Design review of the part built by this model. Coordinates are the model's own, in mm. A direction names the side the tool comes from. Give positions to 0.01 mm unless a question says otherwise; leave off trailing zeros. Loops run counter-clockwise (first coordinate to the right, second up) from the corner with the lowest first, then second, coordinate; pieces in that order, holes last. Notation, with made-up numbers: (50.5, -8) -> (101.5, -8) arc R17 cw to (101.5, 14) -> close; hole circle Ø7 at (-17.5, 6). An arc over 180 degrees is marked (long way). Use a Markdown table: item, result. Add a question column.
1. Add section B-B (x = -83). State the section outline as (y, z) points, and give its area (3 significant figures).
2. To check wall thickness, follow line 1 (X direction, y = 2.5, z = -6); line 2 (Y direction, x = -66, z = -6.5); line 3 (Y direction, x = -9, z = -10). State the ranges of each line that lie inside material, in increasing order.
3. Add section C-C (y = 19). State the section outline as (x, z) points, and give its area (3 significant figures).
4. Add section A-A (z = 3.5). State the section outline as (x, y) points, and give its area (3 significant figures).
5. Draft analysis for pull direction X (two halves, no side actions). For faces 4 (the cylindrical face through (-99.1, 5.07, -20.14)), 5 (the cylindrical face through (-82.85, 11.97, -16.5)), 6 (the flat face through (-22.36, 32.38, 14.82)), state which applies: pulls with the +X half, pulls with the -X half, needs draft (parallel to the pull), parting line crosses it, or undercut.
6. For pin 1 Ø3 at (y, z) = (12, 2.5) entering from -X; pin 2 Ø11 at (x, z) = (-82, -3) entering from +Y; pin 3 Ø1.2 at (y, z) = (11.5, -1.5) entering from +X, all flat-tipped, find the tip position at first contact; note any pin that passes through.
7. Add section D-D (x = -19.5). State the section outline as (y, z) points, and give its area (3 significant figures).
8. For faces 1 (the cylindrical face through (-83.15, 11.97, 16.5)), 2 (the flat face through (-22.36, 29.612, 9.962)), 3 (the flat face through (-90, 12, 0)), list the 3-axis set-ups (+Z, -Z, +X, -X, +Y, -Y) from which the entire face can be reached by the end or side of a thin tool; tool diameter is ignored.
```python
from build123d import *

# Parameters (mm, degrees)
BASE_BLOCK_DEPTH         = 21
SLOT_BOSS_DEPTH          = 4
MOUNTING_START           = -34
MOUNTING_SLOT_DEPTH      = 34
DOVETAIL_GROOVE_55_DEPTH = 464
EDGE_FILLET_R3_R         = 3


with BuildPart() as part:
    # Base Profile Sketch → Base Block (new, symmetric)
    with BuildSketch(Plane.XY):
        Polygon((0, 0), (-100, 0), (-100, 10), (-60, 10), (-60, 31), (-44.102715558, 50.294464164), (0, 22.736028876), align=None)
    extrude(amount=BASE_BLOCK_DEPTH, both=True)

    # Slot Boss Sketch → Slot Boss (add)
    with BuildSketch(Plane(origin=(0, 10, 0), x_dir=(1, 0, 0), z_dir=(0, 1, 0))):
        with BuildLine():
            Line((-90, 9.5), (-90, -9.5))
            ThreePointArc((-90, -9.5), (-83, -16.5), (-76, -9.5))
            Line((-76, -9.5), (-76, 9.5))
            ThreePointArc((-76, 9.5), (-83, 16.5), (-90, 9.5))
        make_face()
        with BuildLine():
            Line((-88, 9.5), (-88, -9.5))
            ThreePointArc((-88, -9.5), (-83, -14.5), (-78, -9.5))
            Line((-78, -9.5), (-78, 9.5))
            ThreePointArc((-78, 9.5), (-83, 14.5), (-88, 9.5))
        make_face(mode=Mode.SUBTRACT)
    extrude(amount=SLOT_BOSS_DEPTH)

    # Mounting Slot Sketch → Mounting Slot (cut)
    with BuildSketch(Plane(origin=(0, 10, 0), x_dir=(1, 0, 0), z_dir=(0, 1, 0)).offset(MOUNTING_START)):
        with BuildLine():
            Line((-88, 9.5), (-88, -9.5))
            ThreePointArc((-88, -9.5), (-83, -14.5), (-78, -9.5))
            Line((-78, -9.5), (-78, 9.5))
            ThreePointArc((-78, 9.5), (-83, 14.5), (-88, 9.5))
        make_face()
    extrude(amount=MOUNTING_SLOT_DEPTH, mode=Mode.SUBTRACT)

    # Dovetail Groove Sketch → Dovetail Groove 55° (cut)
    with BuildSketch(Plane(origin=(-50.952316762, 41.981133327, 0), x_dir=(0, 0, 1), z_dir=(-0.7717785665555229, 0.635891377678218, 0))):
        Polygon((-11.5, 6.439032464), (-8.466266509, 10.771652903), (-21, 10.771652903), (-21, 17.547179775), (21, 17.547179775), (21, 10.771652903), (8.466266509, 10.771652903), (11.5, 6.439032464), align=None)
    extrude(amount=-DOVETAIL_GROOVE_55_DEPTH, mode=Mode.SUBTRACT)

    # Edge Fillet R3
    edge_fillet_r3_edges = [part.edges().sort_by_distance(p)[0] for p in [
        (-100, 5, 21),
        (-100, 5, -21),
    ]]
    fillet(edge_fillet_r3_edges, radius=EDGE_FILLET_R3_R)


solid = part.part
```
Taken from the geometry:
| question | item | result |
|---|---|---|
| 1 | outline | (0, -21) -> (10, -21) -> (10, -16.5) -> (14, -16.5) -> (14, -14.5) -> (0, -14.5) -> close; (0, 14.5) -> (14, 14.5) -> (14, 16.5) -> (10, 16.5) -> (10, 21) -> (0, 21) -> close |
| 1 | area | 146 mm^2 |
| 2 | line 1 | x = -100 to -88, -78 to 0 |
| 2 | line 2 | y = 0 to 10 |
| 2 | line 3 | y = 0 to 15.76, 18.53 to 21.37 |
| 3 | outline | (-60, -21) -> (-6.12, -21) -> (-6.12, -8.47) -> (-12.93, -11.5) -> (-12.93, 11.5) -> (-6.12, 8.47) -> (-6.12, 21) -> (-60, 21) -> close |
| 3 | area | 2,130 mm^2 |
| 4 | outline | (-100, 0) -> (-88, 0) -> (-88, 14) -> (-90, 14) -> (-90, 10) -> (-100, 10) -> close; (-78, 0) -> (0, 0) -> (0, 8.34) -> (-46.86, 46.95) -> (-60, 31) -> (-60, 10) -> (-76, 10) -> (-76, 14) -> (-78, 14) -> close |
| 4 | area | 2,120 mm^2 |
| 5 | face 4 | pulls with the -X half |
| 5 | face 5 | undercut |
| 5 | face 6 | pulls with the +X half |
| 6 | pin 1 | stops at x = -90 |
| 6 | pin 2 | stops at y = 14 |
| 6 | pin 3 | stops at x = -3.1 |
| 7 | outline | (0, -21) -> (30.02, -21) -> (30.02, -8.47) -> (24.41, -11.5) -> (24.41, 11.5) -> (30.02, 8.47) -> (30.02, 21) -> (0, 21) -> close |
| 7 | area | 1,150 mm^2 |
| 8 | face 1 | +Z, +Y |
| 8 | face 2 | none |
| 8 | face 3 | +Z, -Z, -X, +Y |
